Work out the finished part from the listing and answer in its coordinate system (mm). A direction names the side the tool comes from. Round coordinates to 2 decimals unless told otherwise and drop trailing zeros. Loops run counter-clockwise (first coordinate to the right, second up) from the corner with the lowest first, then second, coordinate; pieces in that order, holes last. Notation, with made-up numbers: (54, -15) - (82, -15) arc R31 ccw to (82, 20) - close; hole circle Ø10 at (19.25, -34.5). An arc over 180 degrees is marked (long way). Answer as CSV lines item,"result". Start each with the question number.
Q1. Section A-A on y = 0 is taken. Write down the section's boundary in (x, z).
Q2. The mould has two halves that part along Z. Classify faces 4 (the face through (-35, 23, -72)), 5 (the face through (-42.395, 66.538, 34.608)), 6 (the face through (-48.125, -55.08, 2.232)): +Z half, -Z half, draft (parallel to the pull), parting line (faces both ways), or undercut.
Q3. For faces 1 (the face through (35, 72, 23)), 2 (the face through (1, 61.4, 0)), 3 (the face through (0.252, 66.538, 34.608)), determine the directions among +Z, -Z, +X, -X, +Y, -Y from which every point of the face is accessible in a straight line to the end or side of a thin tool.
Q4. Each of these flat-tipped pins is pushed along its axis until it touches: pin 1 Ø14.5 at (y, z) = (92.5, 0) entering from -X; pin 2 Ø18.5 at (y, z) = (-74.83, 54.37) entering from -X; pin 3 Ø1.5 at (y, z) = (-4.5, 76.5) entering from +X; pin 4 Ø1.5 at (x, y) = (16.5, -5) entering from +Z. Where does it stop, or does it pass through?
Q5. Section B-B on y = 92.5 is taken. Write down the section's boundary in (x, z), then the cut area to 3 significant figures.
Q6. Straight lines are drawn through the part: L1, parallel to X at y = 90, z = -42; L2, parallel to Y at x = 2, z = 0; L3, parallel to Z at x = -27, y = 81. For each, find the intervals that lie inside material, in ascending order. Write a range as [from, to].
Q7. Section C-C on x = 28.5 is taken. Count the separate pieces of the cut face and the enclosed holes in it, then the cut area to 3 significant figures.
Q8. Section D-D on x = 0 is taken. Write down the section's boundary in (y, z).
```python
from build123d import *

# Parameters (mm, degrees)
SKETCH2_R          = 8
CUT_EXTRUDE1_DEPTH = 178.270979012
CIRPATTERN1_COUNT  = 10
SKETCH3_W          = 28
SKETCH3_H          = 61.4
CUT_EXTRUDE2_DEPTH = 185.932420089


with BuildPart() as part:
    # Sketch1 → Revolve1 (revolve)
    with BuildSketch(Plane.XY, mode=Mode.PRIVATE) as revolve1_sk:
        Polygon((-50, 57), (-50, 75), (-35, 75), (-35, 110), (-18, 110), (-18, 75), (18, 75), (18, 110), (35, 110), (35, 75), (50, 75), (50, 57), (48, 55), (-48, 55), align=None)
    revolve(revolve1_sk.sketch.rotate(Axis((-54.276945294, 0, 0), (1, 0, 0)), 90), axis=Axis((-54.276945294, 0, 0), (1, 0, 0)))

    # Sketch2 → Cut-Extrude1 (cut, through all)
    with BuildSketch(Plane.ZY.offset(35)):
        with Locations((0, 92.5)):
            Circle(SKETCH2_R)
    cut_extrude1 = extrude(amount=-CUT_EXTRUDE1_DEPTH, mode=Mode.SUBTRACT)

    # CirPattern1: Cut-Extrude1 ×10 about axis
    cirpattern1_axis = Axis((0, 0, 0), (1, 0, 0))
    for i in range(1, CIRPATTERN1_COUNT):
        add(cut_extrude1.rotate(cirpattern1_axis, i * 360 / CIRPATTERN1_COUNT), mode=Mode.SUBTRACT)

    # Sketch3 → Cut-Extrude2 (cut, through all)
    with BuildSketch(Plane(origin=(50, 0, 0), x_dir=(0, 0, -1), z_dir=(1, 0, 0))):
        with Locations((0, 30.7)):
            Rectangle(SKETCH3_W, SKETCH3_H)
    extrude(amount=-CUT_EXTRUDE2_DEPTH, mode=Mode.SUBTRACT)


solid = part.part
```
Findings:
1,outline,"(-50, -75) - (-35, -75) - (-35, -110) - (-18, -110) - (-18, -75) - (18, -75) - (18, -110) - (35, -110) - (35, -75) - (50, -75) - (50, -57) - (48, -55) - (-48, -55) - (-50, -57) - close; (-50, 57) - (-48, 55) - (48, 55) - (50, 57) - (50, 75) - (35, 75) - (35, 110) - (18, 110) - (18, 75) - (-18, 75) - (-18, 110) - (-35, 110) - (-35, 75) - (-50, 75) - close"
2,face 4,"draft"
2,face 5,"parting line"
2,face 6,"undercut"
3,face 1,"+X"
3,face 2,"+X, -X"
3,face 3,"none"
4,pin 1,"passes through"
4,pin 2,"stops at x = -35"
4,pin 3,"stops at x = 35"
4,pin 4,"stops at z = 74.88"
5,outline,"(-35, -59.53) - (-18, -59.53) - (-18, -8) - (-35, -8) - close; (-35, 8) - (-18, 8) - (-18, 59.53) - (-35, 59.53) - close; (18, -59.53) - (35, -59.53) - (35, -8) - (18, -8) - close; (18, 8) - (35, 8) - (35, 59.53) - (18, 59.53) - close"
5,area,"3,500 mm^2"
6,L1,"x = [-35, -18], [18, 35]"
6,L2,"y = [-75, -55], [61.4, 75]"
6,L3,"z = [-74.42, -59.47], [-49.27, 49.27], [59.47, 74.42]"
7,separate pieces,"1"
7,enclosed holes,"11"
7,area,"26,300 mm^2"
8,outline,"circle Ø150 at (0, 0); hole (53.19, -14) - (61.4, -14) - (61.4, 14) - (53.19, 14) arc R55 ccw (long way) to start"
